Part model, mm, in its own coordinate system. Face numbers are marked on the shaded views. Round coordinates to 2 decimals unless told otherwise and drop trailing zeros. Loops run counter-clockwise (first coordinate to the right, second up) from the corner with the lowest first, then second, coordinate; pieces in that order, holes last.
1) Band-saw the part on C-C, the plane x = 67. Write the cut outline in (y, z).
2) Mould opens along Z. For the marked faces 1, 2 and 3 say: +Z half, -Z half, draft (parallel to the pull), parting line (faces both ways), or undercut.
3) Band-saw the part on A-A, the plane z = 0. Write the cut outline in (x, y).
4) Drop flat-ended pins along their axis: P1, Ø3, axis at x = 73, y = 13, coming from the +Z side; P2, Ø21, axis at y = 6.5, z = 3.5, coming from the -X side; P3, Ø6, axis at x = 94, z = -5.5, coming from the -Y side; P4, Ø25, axis at y = 0, z = 0, coming from the +X side. Give the stop position or say it passes through.
5) Probe line 1 (Y direction, x = 8.25, z = 0); line 2 (X direction, y = -16, z = 12.5); line 3 (Z direction, x = 9, y = 17). List the from-to ranges inside material, lowest first.
from build123d import *

# Parameters (mm, degrees)
SKETCH1_W          = 120
SKETCH1_H          = 30
SKETCH2_R          = 21
CUT_EXTRUDE1_DEPTH = 15
CUT_EXTRUDE2_START = -15
SKETCH4_R          = 21
CUT_EXTRUDE2_DEPTH = 15
SKETCH5_R          = 17.5
CUT_EXTRUDE3_DEPTH = 114.247516529
SKETCH8_R          = 41.443957881
SKETCH8_R_2        = 24
CUT_EXTRUDE4_DEPTH = 128.279220614
CHAMFER1_SIZE      = 1
CHAMFER3_SIZE      = 1


with BuildPart() as part:
    # Sketch1 → Revolve1 (revolve)
    with BuildSketch(Plane.XY, mode=Mode.PRIVATE) as revolve1_sk:
        with Locations((60, 15)):
            Rectangle(SKETCH1_W, SKETCH1_H)
    revolve(revolve1_sk.sketch.rotate(Axis((0, 0, 0), (-1, 0, 0)), 90), axis=Axis((0, 0, 0), (-1, 0, 0)))

    # Sketch2 → Cut-Extrude1 (cut)
    with BuildSketch(Plane.ZY):
        Circle(SKETCH2_R)
    extrude(amount=-CUT_EXTRUDE1_DEPTH, mode=Mode.SUBTRACT)

    # Sketch4 → Cut-Extrude2 (cut)
    with BuildSketch(Plane(origin=(120, 0, 0), x_dir=(0, 0, -1), z_dir=(1, 0, 0)).offset(CUT_EXTRUDE2_START)):
        with Locations(Location((0, 0, 0), (0, 0, 180))):
            Circle(SKETCH4_R)
    extrude(amount=CUT_EXTRUDE2_DEPTH, mode=Mode.SUBTRACT)

    # Sketch5 → Cut-Extrude3 (cut, through all)
    with BuildSketch(Plane(origin=(105, 0, 0), x_dir=(0, 0, -1), z_dir=(1, 0, 0))):
        Circle(SKETCH5_R)
    extrude(amount=-CUT_EXTRUDE3_DEPTH, mode=Mode.SUBTRACT)

    # Sketch8 → Cut-Extrude4 (cut, through all)
    with BuildSketch(Plane.ZY):
        Circle(SKETCH8_R)
        Circle(SKETCH8_R_2, mode=Mode.SUBTRACT)
    extrude(amount=-CUT_EXTRUDE4_DEPTH, mode=Mode.SUBTRACT)

    # Chamfer1
    chamfer1_edges = [part.edges().sort_by_distance(p)[0] for p in [
        (0, 0, -24),
    ]]
    chamfer(chamfer1_edges, length=CHAMFER1_SIZE)

    # Chamfer3
    chamfer3_edges = [part.edges().sort_by_distance(p)[0] for p in [
        (120, 0, -24),
    ]]
    chamfer(chamfer3_edges, length=CHAMFER3_SIZE)


solid = part.part
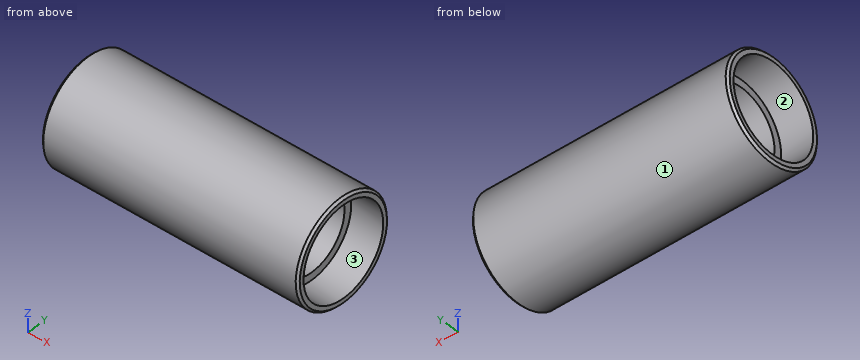
Reported:
1. outline: circle Ø48 at (0, 0); hole circle Ø35 at (0, 0)
2. face 1: parting line
2. face 2: undercut
2. face 3: undercut
3. outline: (0, -23) - (1, -24) - (119, -24) - (120, -23) - (120, -21) - (105, -21) - (105, -17.5) - (15, -17.5) - (15, -21) - (0, -21) - close; (0, 21) - (15, 21) - (15, 17.5) - (105, 17.5) - (105, 21) - (120, 21) - (120, 23) - (119, 24) - (1, 24) - (0, 23) - close
4. P1: stops at z = 21.07
4. P2: stops at x = 15
4. P3: stops at y = -23.87
4. P4: passes through
5. line 1: y = -24 to -21, 21 to 24
5. line 2: x = 15 to 105
5. line 3: z = -16.94 to -12.33, 12.33 to 16.94
